from build123d import *

# Parameters (mm, degrees)
SKETCH_1_W               = 206
SKETCH_1_H               = 145
EXTRUDE_1_DEPTH          = 6
SKETCH_3_R               = 4.5
CUT_EXTRUDE_2_DEPTH      = 127.100158604
SKETCH_4_R               = 22.5
CUT_EXTRUDE_3_DEPTH      = 127.100158604
FILLET_1_R               = 57
HOLE_WIZARD_M6_1_D       = 5
PATTERN_CIRCULAR_1_COUNT = 4
SKETCH_11_R              = 4.5
CUT_EXTRUDE_6_DEPTH      = 127.100158604
FILLET_5_R               = 3


with BuildPart() as part:
    # 草图1 → 凸台-拉伸1 (new body)
    with BuildSketch(Plane.XY):
        Rectangle(SKETCH_1_W, SKETCH_1_H)
    extrude(amount=EXTRUDE_1_DEPTH)

    # 草图3 → 切除-拉伸2 (cut, through all)
    with BuildSketch(Plane.XY.offset(6)):
        with Locations((-88, 55)):
            Circle(SKETCH_3_R)
        with Locations((-48, 55)):
            Circle(SKETCH_3_R)
        with Locations((-88, -62.5)):
            Circle(SKETCH_3_R)
        with Locations((-48, -62.5)):
            Circle(SKETCH_3_R)
    extrude(amount=-CUT_EXTRUDE_2_DEPTH, mode=Mode.SUBTRACT)

    # 草图4 → 切除-拉伸3 (cut, through all)
    with BuildSketch(Plane.XY.offset(6)):
        with Locations((46, 15.5)):
            Circle(SKETCH_4_R)
    extrude(amount=-CUT_EXTRUDE_3_DEPTH, mode=Mode.SUBTRACT)

    # 圆角1
    fillet_1_edges = [part.edges().sort_by_distance(p)[0] for p in [
        (103, 72.5, 3),
    ]]
    fillet(fillet_1_edges, radius=FILLET_1_R)

    # M6 螺纹孔1 (through all)
    with Locations(Plane.XY.offset(6)):
        with Locations((9.230447378, 52.269552622)):
            hole_wizard_m6_1 = Hole(HOLE_WIZARD_M6_1_D / 2)

    # 阵列(圆周)1: M6 螺纹孔1 ×4 about axis
    pattern_circular_1_axis = Axis((46, 15.5, 0), (0, 0, 1))
    for i in range(1, PATTERN_CIRCULAR_1_COUNT):
        add(hole_wizard_m6_1.rotate(pattern_circular_1_axis, i * 360 / PATTERN_CIRCULAR_1_COUNT), mode=Mode.SUBTRACT)

    # 草图11 → 切除-拉伸6 (cut, through all)
    with BuildSketch(Plane.XY.offset(6)):
        with Locations((73, -62.5)):
            Circle(SKETCH_11_R)
    extrude(amount=-CUT_EXTRUDE_6_DEPTH, mode=Mode.SUBTRACT)

    # 圆角5
    fillet_5_edges = [part.edges().sort_by_distance(p)[0] for p in [
        (103, -72.5, 3),
    ]]
    fillet(fillet_5_edges, radius=FILLET_5_R)


solid = part.part
Build history of the part. All positions in model axes, mm. Round coordinates to 2 decimals unless told otherwise and drop trailing zeros. Loops run counter-clockwise (first coordinate to the right, second up) from the corner with the lowest first, then second, coordinate; pieces in that order, holes last. Notation, with made-up numbers: (-30.5, 17.25) -> (-16.5, 17.25) arc R24 cw to (-16.5, 41.25) -> close; hole circle Ø8 at (-14.5, 44.25). An arc over 180 degrees is marked (long way). Use CSV: the item, a comma, the result in double quotes. Start each with the question number.
Q1. Mould opens along Y. For faces 1 (the face through (-92.496, -62.302, 3.042)), 2 (the face through (85.859, 56.246, 3.042)), 3 (the face through (-1, 1, 6)) say: +Y half, -Y half, draft (parallel to the pull), parting line (faces both ways), or undercut.
Q2. Drill centre lines: L1, parallel to Y at x = -88, z = 2.15; L2, parallel to X at y = -63, z = 3.7; L3, parallel to X at y = -64, z = 0.3. Where is each one in solid material? Low to high.
Q3. Saw through at A-A on x = -48. Give the cut face in (y, z), and give its area (3 significant figures).
Q4. Flat gauge pin, fed straight in: pin 1 Ø4.5 at (x, y) = (9.23, -21.27) entering from +Z. Where does the tip first touch, or does it go through?
Q5. Saw through at B-B on y = -62.5. Give the cut face in (x, z).
Q6. Saw through at C-C on x = 73. Give the cut face in (y, z).
Q7. Saw through at D-D on z = 3.4. Count the separate pieces of the cut face and the enclosed holes in it, and give its area (3 significant figures).
Solutions:
1,face 1,"undercut"
1,face 2,"+Y half"
1,face 3,"draft"
2,L1,"y = -72.5 to -67, -58 to 50.5, 59.5 to 72.5"
2,L2,"x = -103 to -92.47, -83.53 to -52.47, -43.53 to 68.53, 77.47 to 103"
2,L3,"x = -103 to -92.24, -83.76 to -52.24, -43.76 to 68.76, 77.24 to 103"
3,outline,"(-72.5, 0) -> (-67, 0) -> (-67, 6) -> (-72.5, 6) -> close; (-58, 0) -> (50.5, 0) -> (50.5, 6) -> (-58, 6) -> close; (59.5, 0) -> (72.5, 0) -> (72.5, 6) -> (59.5, 6) -> close"
3,area,"762 mm^2"
4,pin 1,"passes through"
5,outline,"(-103, 0) -> (-92.5, 0) -> (-92.5, 6) -> (-103, 6) -> close; (-83.5, 0) -> (-52.5, 0) -> (-52.5, 6) -> (-83.5, 6) -> close; (-43.5, 0) -> (68.5, 0) -> (68.5, 6) -> (-43.5, 6) -> close; (77.5, 0) -> (103, 0) -> (103, 6) -> (77.5, 6) -> close"
6,outline,"(-72.5, 0) -> (-67, 0) -> (-67, 6) -> (-72.5, 6) -> close; (-58, 0) -> (65.7, 0) -> (65.7, 6) -> (-58, 6) -> close"
7,separate pieces,"1"
7,enclosed holes,"10"
7,area,"27,200 mm^2"
